Could you check a few things on this model? Use its own coordinates, in mm. Face numbers are marked on the shaded views. A direction names the side the tool comes from. Coordinates: 2 decimals unless noted, no trailing zeros. Order: outer loops, then holes, each group sorted by start corner. A loop starts at its lowest first (then second) coordinate and runs counter-clockwise, first axis right, second up. Notation, with made-up numbers: (62, 85.25) - (91, 85.25) arc R24 ccw to (91, 119.25) - close; hole circle Ø7 at (-26.75, 25). An arc over 180 degrees is marked (long way). One line per item, written item: value.
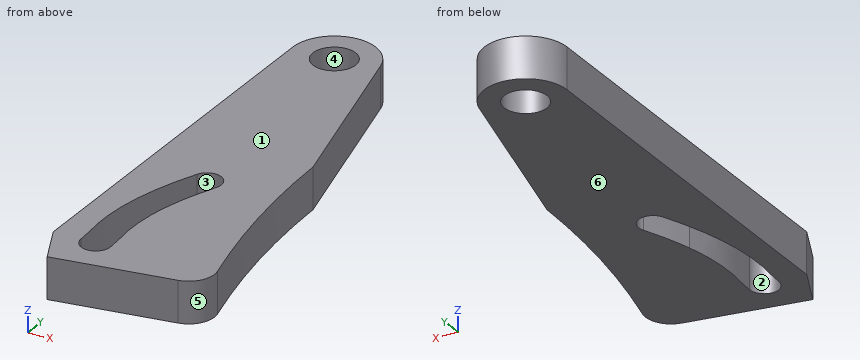
from build123d import *

# Parameters (mm, degrees)
SKETCH_1_R      = 1.55
EXTRUDE_1_DEPTH = 3


with BuildPart() as part:
    # 草图1 (on Front Plane) → 凸台-拉伸1 (new body)
    with BuildSketch(Plane.XY):
        with BuildLine():
            Line((3.816218697, 0.711369777), (0.741076539, 14.191366792))
            ThreePointArc((0.741076539, 14.191366792), (-2.49053861, 16.508405149), (-5.183215516, 13.582402021))
            Line((-5.183215516, 13.582402021), (-5.732788153, -14.705577537))
            Line((-5.732788153, -14.705577537), (-4.408096335, -17.704776028))
            Line((-4.408096335, -17.704776028), (4.127837654, -16.252589359))
            ThreePointArc((4.127837654, -16.252589359), (5.371423242, -15.437528643), (5.619036958, -13.971405684))
            ThreePointArc((5.619036958, -13.971405684), (4.268609288, -6.685150501), (3.816218697, 0.711369777))
        make_face()
        with Locations((-2.183781514, 13.524129678)):
            Circle(SKETCH_1_R, mode=Mode.SUBTRACT)
        with BuildLine():
            ThreePointArc((-3.783386383, -14.657279108), (-2.707701661, -15.680950138), (-1.684030631, -14.605265415))
            add(Edge.make_bspline(
                [(-1.684030631, -14.605265415), (-1.698385943, -14.230913496), (-1.690645088, -13.65109076), (-1.790811076, -12.90815818), (-1.819576713, -12.363575922), (-1.822848669, -11.844967012), (-1.807105928, -11.320378821), (-1.768151471, -10.788389789), (-1.707646295, -10.25185083), (-1.625402268, -9.709964922), (-1.486001031, -8.974109842), (-1.351215721, -8.423808693), (-1.249236023, -8.057041386)],
                knots=[0, 0, 0, 0, 0.170354994, 0.26229743, 0.340043602, 0.417823563, 0.497759338, 0.578301179, 0.659976625, 0.742887413, 0.827131807, 1, 1, 1, 1], degree=3))
            add(Edge.make_bspline(
                [(0.03013882, -4.613074169), (-0.143309735, -4.996054164), (-0.391510935, -5.572837816), (-0.692509933, -6.347460357), (-0.964714861, -7.105557392), (-1.143447826, -7.676581339), (-1.249236023, -8.057041386)],
                knots=[0, 0, 0, 0, 0.342979707, 0.512099324, 0.677879853, 1, 1, 1, 1], degree=3))
            ThreePointArc((0.03013882, -4.613074169), (-0.488256217, -3.213540285), (-1.882444762, -3.746144084))
            add(Edge.make_bspline(
                [(-3.783386383, -14.657279108), (-3.799290999, -14.2981548), (-3.786309002, -13.774144994), (-3.886484574, -13.055813522), (-3.915903208, -12.486133418), (-3.923833984, -11.87345296), (-3.906620769, -11.257653943), (-3.849073975, -10.432184554), (-3.741043656, -9.603680421), (-3.586380227, -8.77634916), (-3.446679883, -8.151733856), (-3.28447898, -7.525898679), (-3.10051603, -6.898880381), (-2.895571139, -6.270661953), (-2.670469593, -5.64113868), (-2.342560405, -4.794442901), (-2.072047563, -4.164799113), (-1.882444762, -3.746144084)],
                knots=[0, 0, 0, 0, 0.096210271, 0.139297547, 0.1935541, 0.248477319, 0.302979464, 0.358078206, 0.469497102, 0.525932365, 0.582904263, 0.640455034, 0.69862477, 0.757451361, 0.816970378, 0.877214945, 1, 1, 1, 1], degree=3))
        make_face(mode=Mode.SUBTRACT)
    extrude(amount=EXTRUDE_1_DEPTH)


solid = part.part
Item 1: I'm going to push flat-ended pins straight in: pin 1 Ø1.5 at (x, y) = (4.5, 3.5) entering from +Z; pin 2 Ø1 at (x, z) = (2.5, 2) entering from -Y. Where does each tip first touch, or does it pass through?
Conclusion:
pin 1: through
pin 2: y = -16.61
Item 2: I want a section at C-C on x = 3.5. Please give me the cut outline in (y, z).
Conclusion:
outline: (-16.36, 0) - (2.1, 0) - (2.1, 3) - (-16.36, 3) - close
Item 3: If I drill on probe 1 along X at (y, z) = (-14.5, 1.85); probe 2 along X at (y, z) = (-10.5, 2.45); probe 3 along Y at (x, z) = (0, 1.3), over which ranges is the centre line in solid material (lowest first)?
Conclusion:
probe 1: -5.73 to -3.79, -1.69 to 5.67
probe 2: -5.65 to -3.85, -1.73 to 4.86
probe 3: -16.95 to -4.68, -3.67 to 15.58
Item 4: I want a section at B-B on y = 5. Please give me the cut outline in (x, z).
Conclusion:
outline: (-5.35, 0) - (2.84, 0) - (2.84, 3) - (-5.35, 3) - close
Item 5: I want a section at A-A on z = 2.2. Give the number of separate pieces and of enclosed holes in the cut face, then the cut area to 3 significant figures.
Conclusion:
separate pieces: 1
enclosed holes: 2
area: 257 mm²
Item 6: For the marked faces 1 and 2, which set-ups out of +Z, -Z, +X, -X, +Y, -Y let a thin tool reach every point of the face, with its end or its side?
Conclusion:
face 1: +Z, +X, -X, +Y, -Y
face 2: +Z, -Z
Item 7: Thinking about a two-plate mould opening in Y: for the marked faces 3, 4, 5 and 6, which applies, pulls with the +Y half, pulls with the -Y half, needs draft (parallel to the pull), parting line crosses it, or undercut?
Conclusion:
face 3: undercut
face 4: undercut
face 5: parting line crosses it
face 6: needs draft
